from build123d import *

# Parameters (mm, degrees)
BASE_PLATE_PROFILE_W      = 100
BASE_PLATE_PROFILE_H      = 60
BASE_PLATE_2_5MM_DEPTH    = 2.5
RIM_WALL_PROFILE_W        = 100
RIM_WALL_PROFILE_H        = 60
RIM_WALL_PROFILE_W_2      = 95
RIM_WALL_PROFILE_H_2      = 56
RIM_WALL_7_5MM_DEPTH      = 7.5
CORNER_GUSSETS_20MM_DEPTH = 20


with BuildPart() as part:
    # Base Plate Profile → Base Plate 2.5mm (new body)
    with BuildSketch(Plane.XY):
        with Locations((50, 30)):
            Rectangle(BASE_PLATE_PROFILE_W, BASE_PLATE_PROFILE_H)
    extrude(amount=BASE_PLATE_2_5MM_DEPTH)

    # Rim Wall Profile → Rim Wall 7.5mm (add)
    with BuildSketch(Plane.XY.offset(2.5)):
        with Locations((50, 30)):
            Rectangle(RIM_WALL_PROFILE_W, RIM_WALL_PROFILE_H)
        with Locations((50, 29.5)):
            Rectangle(RIM_WALL_PROFILE_W_2, RIM_WALL_PROFILE_H_2, mode=Mode.SUBTRACT)
    extrude(amount=RIM_WALL_7_5MM_DEPTH)

    # Corner Gusset Profile → Corner Gussets 20mm (add)
    with BuildSketch(Plane.XY.offset(2.5)):
        Polygon((2.5, 57.5), (22.5, 57.5), (2.5, 37.5), align=None)
        Polygon((2.5, 1.5), (22.5, 1.5), (2.5, 21.5), align=None)
        Polygon((97.5, 57.5), (77.5, 57.5), (97.5, 37.5), align=None)
        Polygon((97.5, 1.5), (77.5, 1.5), (97.5, 21.5), align=None)
    extrude(amount=CORNER_GUSSETS_20MM_DEPTH)


solid = part.part
Work out the finished part from the listing and answer in its coordinate system (mm). A direction names the side the tool comes from. Round coordinates to 2 decimals unless told otherwise and drop trailing zeros. Write each loop counter-clockwise with the first axis right and the second up, starting at its lowest first coordinate (ties: lowest second). Pieces come first, ordered by that corner, then holes. Notation, with made-up numbers: (-25, 34) -> (-19, 34) arc R24 cw to (-19, 62) -> close; hole circle Ø2 at (50.25, -25.75). An arc over 180 degrees is marked (long way). Write each question's results on one line, items separated by ' | '.
Item 1: A cutting plane is placed at D-D, the plane x = 48.5. Determine the outline of the cut face in (y, z).
Result set:
outline: (0, 0) -> (60, 0) -> (60, 10) -> (57.5, 10) -> (57.5, 2.5) -> (1.5, 2.5) -> (1.5, 10) -> (0, 10) -> close
Item 2: A cutting plane is placed at C-C, the plane z = 14.5. Determine the outline of the cut face in (x, y), plus the area to 3 significant figures.
Result set:
outline: (2.5, 1.5) -> (22.5, 1.5) -> (2.5, 21.5) -> close; (2.5, 37.5) -> (22.5, 57.5) -> (2.5, 57.5) -> close; (77.5, 1.5) -> (97.5, 1.5) -> (97.5, 21.5) -> close; (77.5, 57.5) -> (97.5, 37.5) -> (97.5, 57.5) -> close | area: 800 mm^2
Item 3: Which of the six approach directions +Z, -Z, +X, -X, +Y, -Y give full straight-line access (tool end or side, diameter ignored) to faces 1 (the face through (50, 1.5, 6)), 2 (the face through (97.5, 47, 16)), 3 (the face through (2.5, 47, 16)), 4 (the face through (88, 1.5, 16)), 5 (the face through (12, 57.5, 16))?
Result set:
face 1: +Z | face 2: +Z, +X, +Y, -Y | face 3: +Z, -X, +Y, -Y | face 4: +Z, +X, -X, -Y | face 5: +Z, +X, -X, +Y
Item 4: A cutting plane is placed at B-B, the plane y = 46.5. Determine the outline of the cut face in (x, z).
Result set:
outline: (0, 0) -> (100, 0) -> (100, 10) -> (97.5, 10) -> (97.5, 22.5) -> (88.5, 22.5) -> (88.5, 2.5) -> (11.5, 2.5) -> (11.5, 22.5) -> (2.5, 22.5) -> (2.5, 10) -> (0, 10) -> close
Item 5: Flat-ended cylindrical pins translate along their axes: P1, Ø1.5, axis at y = 15, z = 16.5, coming from the -X side; P2, Ø17, axis at x = 64.5, y = 30, coming from the +Z side; P3, Ø10, axis at x = 86, z = 16, coming from the -Y side. Find the tip coordinate at first contact, or state that the pin passes through.
Result set:
P1: x = 2.5 | P2: z = 2.5 | P3: y = 1.5
Item 6: A cutting plane is placed at A-A, the plane z = 5.5. Determine the outline of the cut face in (x, y), plus the area to 3 significant figures.
Result set:
outline: (0, 0) -> (100, 0) -> (100, 60) -> (0, 60) -> close; hole (2.5, 21.5) -> (22.5, 1.5) -> (77.5, 1.5) -> (97.5, 21.5) -> (97.5, 37.5) -> (77.5, 57.5) -> (22.5, 57.5) -> (2.5, 37.5) -> close | area: 1,480 mm^2
Item 7: Find the intervals of material crossed by line 1 along Y through (x, z) = (40, 7.5); line 2 along Z through (x, y) = (73.5, 7); line 3 along Y through (x, z) = (12, 7), in increasing order. Write a range as [from, to].
Result set:
line 1: [0, 1.5], [57.5, 60] | line 2: [0, 2.5] | line 3: [0, 12], [47, 60]
Item 8: The mould has two halves that part along X. Classify faces 6 (the face through (92, 52, 22.5)), 7 (the face through (0, 30, 5)), 8 (the face through (50, 57.5, 6)): +X half, -X half, draft (parallel to the pull), parting line (faces both ways), or undercut.
Result set:
face 6: draft | face 7: -X half | face 8: undercut
